from build123d import *

# Parameters (mm, degrees)
CIRPATTERN1_COUNT            = 12
F_0_17_0_17_DIAMETER_HOLE1_D = 17.5
CIRPATTERN2_COUNT            = 18
M16_TAPPED_HOLE1_D           = 14
M16_TAPPED_HOLE1_DEPTH       = 35
M16_TAPPED_HOLE1_TIP         = 4.206024333


with BuildPart() as part:
    # Sketch1 → Revolve1 (revolve)
    with BuildSketch(Plane.XY, mode=Mode.PRIVATE) as revolve1_sk:
        with BuildLine():
            Line((-157, 0), (-175, 0))
            Line((-175, 0), (-175, 7.708741574))
            ThreePointArc((-175, 7.708741574), (-166.158424343, 19.100823753), (-177.2, 28.376415566))
            Line((-177.2, 28.376415566), (-177.2, 31.9))
            Line((-177.2, 31.9), (-167, 31.9))
            Line((-167, 31.9), (-167, 40))
            Line((-167, 40), (-149, 40))
            Line((-149, 40), (-149, 35))
            Line((-149, 35), (-121.5, 35))
            Line((-121.5, 35), (-121.5, 10))
            Line((-121.5, 10), (-157, 10))
            Line((-157, 10), (-157, 0))
        make_face()
    revolve(revolve1_sk.sketch.rotate(Axis((0, 22.704798349, 0), (0, 1, 0)), 270), axis=Axis((0, 22.704798349, 0), (0, 1, 0)))

    # Sketch2 → M10x1.0 Tapped Hole1 (revolve, cut)
    with BuildSketch(Plane(origin=(-160, 40, 0), x_dir=(0, 0, 1), z_dir=(1, 0, 0))):
        Polygon((0, 0), (0, 23.703872786), (4.5, 21), (4.5, 0), align=None)
    m10x1_0_tapped_hole1 = revolve(axis=Axis((-160, 46.35, 0), (0, -1, 0)), mode=Mode.SUBTRACT)

    # CirPattern1: M10x1.0 Tapped Hole1 ×12 about axis
    cirpattern1_axis = Axis((0, 0, 0), (0, 1, 0))
    for i in range(1, CIRPATTERN1_COUNT):
        add(m10x1_0_tapped_hole1.rotate(cirpattern1_axis, i * 360 / CIRPATTERN1_COUNT), mode=Mode.SUBTRACT)

    # Ø0.17 (0.17) Diameter Hole1 (through all)
    with Locations(Plane(origin=(0, 35, 0), x_dir=(-1, 0, 0), z_dir=(0, 1, 0))):
        with Locations((0, -135.5)):
            f_0_17_0_17_diameter_hole1 = Hole(F_0_17_0_17_DIAMETER_HOLE1_D / 2)

    # CirPattern2: Ø0.17 (0.17) Diameter Hole1 ×18 about axis
    cirpattern2_axis = Axis((0, 0, 0), (0, 1, 0))
    for i in range(1, CIRPATTERN2_COUNT):
        add(f_0_17_0_17_diameter_hole1.rotate(cirpattern2_axis, i * 360 / CIRPATTERN2_COUNT), mode=Mode.SUBTRACT)

    # M16 Tapped Hole1
    with Locations(Plane(origin=(0, 35, 0), x_dir=(-1, 0, 0), z_dir=(0, 1, 0))):
        with Locations((135.5, 0), (-135.5, 0)):
            Hole(M16_TAPPED_HOLE1_D / 2, depth=M16_TAPPED_HOLE1_DEPTH)
            with Locations((0, 0, -(M16_TAPPED_HOLE1_DEPTH + M16_TAPPED_HOLE1_TIP / 2))):  # 118° drill point
                Cone(0, M16_TAPPED_HOLE1_D / 2, M16_TAPPED_HOLE1_TIP, mode=Mode.SUBTRACT)


solid = part.part
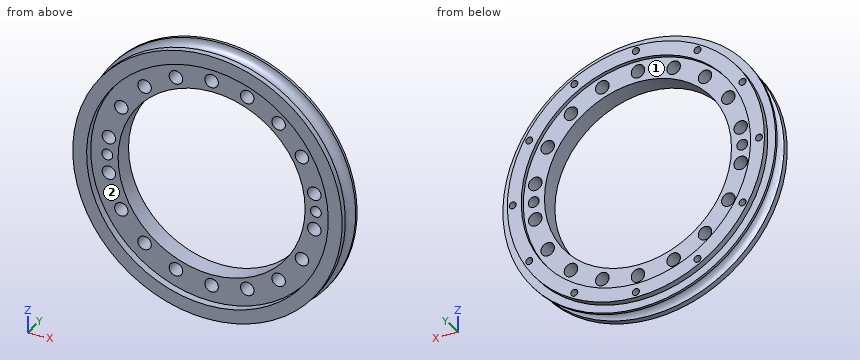
The model under review builds one solid part; all positions refer to its coordinate system, in mm. Face numbers are marked on the shaded views. A direction names the side the tool comes from. Round coordinates to 2 decimals unless told otherwise and drop trailing zeros. Write item = value, one per line. Start each with the question number.
Item 1: For the marked faces 1 and 2, list the 3-axis set-ups (+Z, -Z, +X, -X, +Y, -Y) from which the entire face can be reached by the end or side of a thin tool; tool diameter is ignored.
Item 2: Take a section at A-A on z = -70.5. Count the separate pieces of the cut face and the enclosed holes in it, plus the area to 3 significant figures.
Item 3: To check wall thickness, follow L1, parallel to Z at x = -136, y = 36.5; L2, parallel to X at y = 17, z = 99; L3, parallel to X at y = 23, z = -79.5. State the ranges of each line that lie inside material, in increasing order.
Item 4: Insertion check: pin 1 (1 mm diameter, centred on x = -78, y = 12, fed in from +Z); pin 2 (20 mm diameter, centred on x = -46.34, z = -127.33, fed in from +Y); pin 3 (6 mm diameter, centred on x = 85.5, y = 15, fed in from -Z). Each pin has a flat end and moves straight along its axis. Give the tip position at first contact, or say it passes through.
Result:
q1.face_1 = +Y
q1.face_2 = -Y
q2.separate_pieces = 4
q2.enclosed_holes = 0
q2.area = 2,490 mm²
q3.L1 = -96.92 to -83.7, -76.3 to -60.87, 60.87 to 76.3, 83.7 to 96.92
q3.L2 = -133.43 to -94.41, -79.78 to -70.44, 70.44 to 79.78, 94.41 to 133.43
q3.L3 = -147.3 to -143.04, -134.09 to -91.88, 91.88 to 134.09, 143.04 to 147.3
q4.pin_1 = 149.3
q4.pin_2 = 35
q4.pin_3 = -145.22
